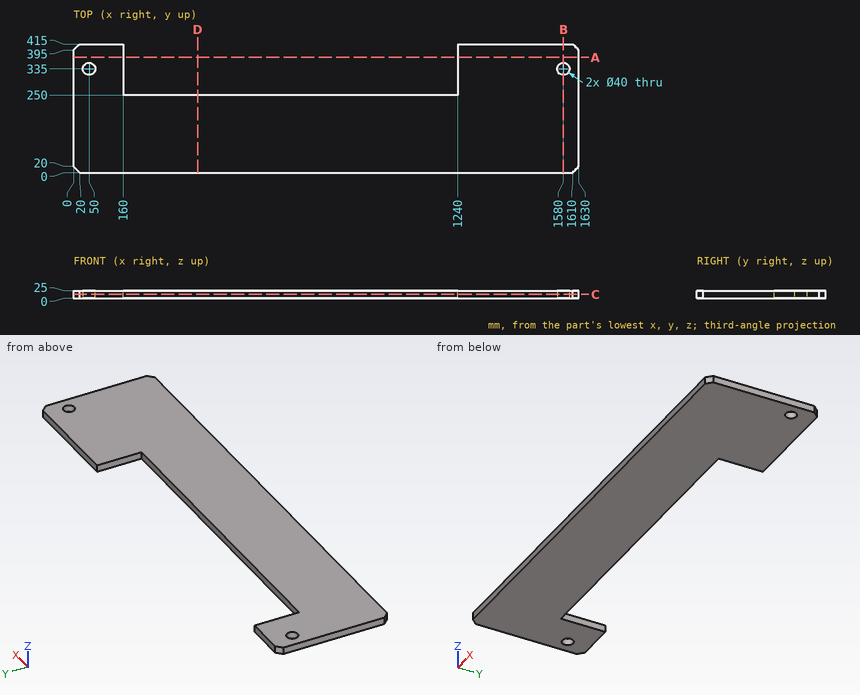
Check sheet for the drawn part. Datum: minimum x, y, z corner. Units: mm. Round coordinates to 2 decimals unless told otherwise and drop trailing zeros. Order: outer loops, then holes, each group sorted by start corner. A loop starts at its lowest first (then second) coordinate and runs counter-clockwise, first axis right, second up. Notation, with made-up numbers: (54, 37.25) -> (102, 37.25) arc R20 cw to (102, 74.25) -> close; hole circle Ø7 at (8.25, 51.5). An arc over 180 degrees is marked (long way). Return JSON: item names as keys, results as strings. Group by question number.
Q1. Section check D-D, the plane x = 400. Record the boundary of the cut face in (y, z).
Q2. Gauge pin test, flat ends, axial feed: pin 1 (24 mm diameter, centred on x = 50, y = 335, fed in from -Z) (3 decimals); pin 2 (7.5 mm diameter, centred on x = 920.5, z = 7, fed in from +Y). Record the tip position at first contact, or that the pin passes through.
Q3. Section check A-A, the plane y = 372. Record the boundary of the cut face in (x, z), plus the area to 4 significant figures.
Q4. Section check C-C, the plane z = 13.25. Record the boundary of the cut face in (x, y).
Q5. Material ranges on probe 1 along X at (y, z) = (335, 8.75); probe 2 along Y at (x, z) = (1580, 16.5); probe 3 along X at (y, z) = (277, 13.5), recorded low to high. Write a range as from..to.
Q6. Section check B-B, the plane x = 1580. Record the boundary of the cut face in (y, z).
Numbers:
{
 "1": {"outline": "(0, 0) -> (250, 0) -> (250, 25) -> (0, 25) -> close"},
 "2": {"pin 1": "through", "pin 2": "y = 250"},
 "3": {"outline": "(0, 0) -> (160, 0) -> (160, 25) -> (0, 25) -> close; (1240, 0) -> (1630, 0) -> (1630, 25) -> (1240, 25) -> close", "area": "13,750 mm^2"},
 "4": {"outline": "(0, 20) -> (20, 0) -> (1610, 0) -> (1630, 20) -> (1630, 395) -> (1610, 415) -> (1240, 415) -> (1240, 250) -> (160, 250) -> (160, 415) -> (20, 415) -> (0, 395) -> close; hole circle Ø40 at (50, 335); hole circle Ø40 at (1580, 335)"},
 "5": {"probe 1": "0..30, 70..160, 1240..1560, 1600..1630", "probe 2": "0..315, 355..415", "probe 3": "0..160, 1240..1630"},
 "6": {"outline": "(0, 0) -> (315, 0) -> (315, 25) -> (0, 25) -> close; (355, 0) -> (415, 0) -> (415, 25) -> (355, 25) -> close"}
}
